Read the model definition and answer for the solid it produces. Units are mm, in the model's axes. Face numbers are marked on the shaded views. A direction names the side the tool comes from. Coordinates: 2 decimals unless noted, no trailing zeros. Order: outer loops, then holes, each group sorted by start corner. A loop starts at its lowest first (then second) coordinate and runs counter-clockwise, first axis right, second up.
```python
from build123d import *

# Parameters (mm, degrees)
STEPPED_CRADLE_BLOCK_65_DEPTH = 65
RAISED_BOSS_SKETCH_W          = 19.460384675
RAISED_BOSS_SKETCH_H          = 51
RAISED_BOSS_DEPTH             = 26
CRADLE_SLOT_SKETCH_W          = 51
CRADLE_SLOT_SKETCH_H          = 51
CRADLE_SLOT_CUT_DEPTH         = 41
CENTER_HOLE_SKETCH_R          = 20
CENTER_HOLE_40_DEPTH          = 41
FRONT_RELIEF_SKETCH_R         = 11.472679984
FRONT_RELIEF_SKETCH_R_2       = 11.491831568
FRONT_RELIEF_CUT_DEPTH        = 41


with BuildPart() as part:
    # Stepped Cradle Profile Sketch → Stepped Cradle Block 65 (new body)
    with BuildSketch(Plane.XY):
        Polygon((-42.445795816, 0), (-42.445795816, 6), (-50.960384675, 6), (-50.960384675, 22), (-62.5, 22), (-62.5, 35), (-50.960384675, 35), (-50.960384675, 51), (-44.960384675, 51), (-8.945795816, 25), (8.945795816, 25), (44.960384675, 51), (50.960384675, 51), (50.960384675, 35), (62.5, 35), (62.5, 22), (50.960384675, 22), (50.960384675, 6), (42.445795816, 6), (42.445795816, 0), (8.945795816, 0), (-8.945795816, 0), align=None)
    extrude(amount=-STEPPED_CRADLE_BLOCK_65_DEPTH)

    # Raised Boss Sketch → Raised Boss (add)
    with BuildSketch(Plane(origin=(0, 25, 0), x_dir=(1, 0, 0), z_dir=(0, 1, 0))):
        with Locations((-35.230192338, 32.5)):
            Rectangle(RAISED_BOSS_SKETCH_W, RAISED_BOSS_SKETCH_H)
        with Locations((35.230192338, 32.5)):
            Rectangle(RAISED_BOSS_SKETCH_W, RAISED_BOSS_SKETCH_H)
    extrude(amount=RAISED_BOSS_DEPTH)

    # Cradle Slot Sketch → Cradle Slot Cut (cut)
    with BuildSketch(Plane(origin=(0, 25, 0), x_dir=(1, 0, 0), z_dir=(0, 1, 0))):
        with Locations((0, 32.5)):
            Rectangle(CRADLE_SLOT_SKETCH_W, CRADLE_SLOT_SKETCH_H)
    extrude(amount=CRADLE_SLOT_CUT_DEPTH, mode=Mode.SUBTRACT)

    # Center Hole Sketch → Center Hole Ø40 (cut)
    with BuildSketch(Plane(origin=(0, 25, 0), x_dir=(1, 0, 0), z_dir=(0, 1, 0))):
        with Locations(Location((0, 32.5, 0), (0, 0, 270))):
            Circle(CENTER_HOLE_SKETCH_R)
    extrude(amount=-CENTER_HOLE_40_DEPTH, mode=Mode.SUBTRACT)

    # Front Relief Sketch → Front Relief Cut (cut)
    with BuildSketch(Plane(origin=(0, 35, 0), x_dir=(1, 0, 0), z_dir=(0, 1, 0))):
        with Locations((62.5, 32.5)):
            Circle(FRONT_RELIEF_SKETCH_R)
        with Locations((-62.5, 32.5)):
            Circle(FRONT_RELIEF_SKETCH_R_2)
    extrude(amount=-FRONT_RELIEF_CUT_DEPTH, mode=Mode.SUBTRACT)


solid = part.part
```
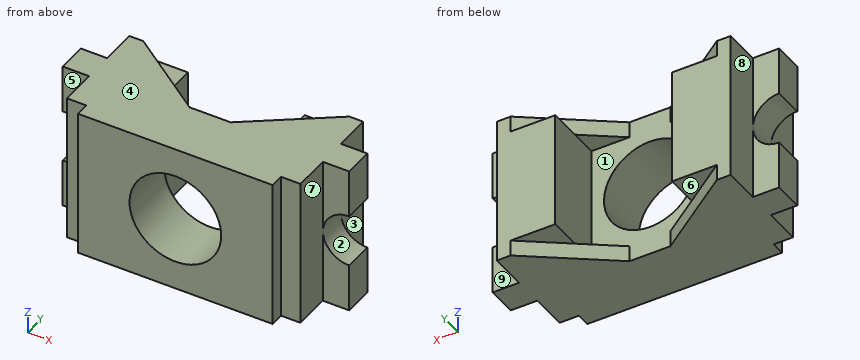
1) Determine the mould class of the marked faces 1, 2, 3 and 4 for opening direction Z: pulls with the +Z half, pulls with the -Z half, needs draft (parallel to the pull), parting line crosses it, or undercut.
A:
face 1: undercut
face 2: undercut
face 3: needs draft
face 4: pulls with the +Z half
2) A cutting plane is placed at C-C, the plane y = 11.5. Determine the outline of the cut face in (x, z).
A:
outline: (-50.96, -65) - (50.96, -65) - (50.96, 0) - (-50.96, 0) - close; hole circle Ø40 at (0, -32.5)
3) Which of the six approach directions +Z, -Z, +X, -X, +Y, -Y give full straight-line access (tool end or side, diameter ignored) to the marked faces 5, 6, 7, 8 and 9?
A:
face 5: +Z, -Z, -X, -Y
face 6: -Z, +Y
face 7: +Z, -Z, +X, -Y
face 8: +Z, -Z, -X, +Y
face 9: +Z, -Z, +X, +Y
4) A cutting plane is placed at A-A, the plane x = 0. Determine the outline of the cut face in (y, z).
A:
outline: (0, -65) - (25, -65) - (25, -52.5) - (0, -52.5) - close; (0, -12.5) - (25, -12.5) - (25, 0) - (0, 0) - close
5) Straight lines are drawn through the part: line 1 (X direction, y = 10.75, z = -32.5); line 2 (X direction, y = 40, z = -13.5); line 3 (Y direction, x = -21, z = -27). For each, find the intervals that lie inside material, in ascending order.
A:
line 1: x = -50.96 to -20, 20 to 50.96
line 2: x = -50.96 to -25.5, 25.5 to 50.96
line 3: y = 0 to 25
6) Flat-ended cylindrical pins translate along their axes: pin 1 Ø6 at (x, z) = (-56.5, -18) entering from +Y; pin 2 Ø13 at (y, z) = (31.5, -25) entering from -X; pin 3 Ø5 at (y, z) = (2.5, -32.5) entering from -X; pin 4 Ø8 at (y, z) = (5.5, -10.5) entering from -X. Find the tip coordinate at first contact, or state that the pin passes through.
A:
pin 1: stops at y = 35
pin 2: stops at x = -62.5
pin 3: stops at x = -42.45
pin 4: stops at x = -50.96
7) A cutting plane is placed at B-B, the plane z = -18. Determine the outline of the cut face in (x, y).
A:
outline: (-62.5, 22) - (-50.96, 22) - (-50.96, 6) - (-42.45, 6) - (-42.45, 0) - (-13.77, 0) - (-13.77, 25) - (-25.5, 25) - (-25.5, 51) - (-50.96, 51) - (-50.96, 35) - (-62.5, 35) - close; (13.77, 0) - (42.45, 0) - (42.45, 6) - (50.96, 6) - (50.96, 22) - (62.5, 22) - (62.5, 35) - (50.96, 35) - (50.96, 51) - (25.5, 51) - (25.5, 25) - (13.77, 25) - close
8) A cutting plane is placed at D-D, the plane y = 46.5. Determine the outline of the cut face in (x, z), and give its area (3 significant figures).
A:
outline: (-50.96, -65) - (-38.73, -65) - (-38.73, -58) - (-25.5, -58) - (-25.5, -7) - (-38.73, -7) - (-38.73, 0) - (-50.96, 0) - close; (25.5, -58) - (38.73, -58) - (38.73, -65) - (50.96, -65) - (50.96, 0) - (38.73, 0) - (38.73, -7) - (25.5, -7) - close
area: 2,940 mm2
